from build123d import *

# Parameters (mm, degrees)
SKETCH_1_W          = 90
SKETCH_1_H          = 80
EXTRUDE_1_DEPTH     = 60
SKETCH_2_R          = 6.2
CUT_EXTRUDE_1_DEPTH = 80


with BuildPart() as part:
    # 草图1 → 凸台-拉伸1 (new, symmetric)
    with BuildSketch(Plane.XY):
        Rectangle(SKETCH_1_W, SKETCH_1_H)
    extrude(amount=EXTRUDE_1_DEPTH, both=True)

    # 草图2 → 切除-拉伸1 (cut, symmetric)
    with BuildSketch(Plane.XY):
        Circle(SKETCH_2_R)
    extrude(amount=CUT_EXTRUDE_1_DEPTH, both=True, mode=Mode.SUBTRACT)


solid = part.part
Verification items for the finished model (mm, model axes). Coordinates: 2 decimals unless noted, no trailing zeros. Write each loop counter-clockwise with the first axis right and the second up, starting at its lowest first coordinate (ties: lowest second). Pieces come first, ordered by that corner, then holes. Notation, with made-up numbers: M 72.5,76 L 123.5,76 A11 ccw 123.5,84 Z; hole C 49,-31.5 d8. An arc over 180 degrees is marked long. One line per question, with ' | ' between items.
1) Depth check by flat-ended pin: pin 1 Ø10 at (x, y) = (0, 0) entering from +Z. Enter the tip coordinate at first touch or a pass-through.
Solutions:
pin 1: through
2) Material ranges on L1, parallel to Y at x = 0, z = -31; L2, parallel to Y at x = -1, z = -46; L3, parallel to X at y = 3, z = 34, recorded low to high.
Solutions:
L1: -40 to -6.2, 6.2 to 40 | L2: -40 to -6.12, 6.12 to 40 | L3: -45 to -5.43, 5.43 to 45
3) Release check for a two-part mould opening along Y. For faces 1 (the face through (-1, -40, 1)), 2 (the face through (-1, 40, 1)), 3 (the face through (2.86, -5.5, 0.84)), 4 (the face through (-45, -1, 1)) record: +Y half, -Y half, draft (parallel to the pull), parting line (faces both ways), or undercut.
Solutions:
face 1: -Y half | face 2: +Y half | face 3: undercut | face 4: draft
4) Sectioned sample at C-C on z = 48. Record the cut outline in (x, y).
Solutions:
outline: M -45,-40 L 45,-40 L 45,40 L -45,40 Z; hole C 0,0 d12.4
5) Sectioned sample at A-A on y = 0. Record the cut outline in (x, z), then the cut area to 3 significant figures.
Solutions:
outline: M -45,-60 L -6.2,-60 L -6.2,60 L -45,60 Z; M 6.2,-60 L 45,-60 L 45,60 L 6.2,60 Z | area: 9,310 mm^2
6) Sectioned sample at B-B on x = 0. Record the cut outline in (y, z).
Solutions:
outline: M -40,-60 L -6.2,-60 L -6.2,60 L -40,60 Z; M 6.2,-60 L 40,-60 L 40,60 L 6.2,60 Z
